Here's how the part is built. I have some questions about the finished solid (model axes, mm). Face numbers are marked on the shaded views. Coordinates: 2 decimals unless noted, no trailing zeros. Write each loop counter-clockwise with the first axis right and the second up, starting at its lowest first coordinate (ties: lowest second). Pieces come first, ordered by that corner, then holes. Notation, with made-up numbers: M -13.75,6.25 L 16.25,6.25 A36 cw 16.25,42.25 Z; hole C 41.5,58 d6. An arc over 180 degrees is marked long. Use one line per item in the form item = value. Start each with the question number.
1. I want a section at C-C, the plane z = 24.75. List the corners of the cut face in (x, y) for me.
2. I want a section at A-A, the plane x = -16. List the corners of the cut face in (y, z) for me.
3. Thinking about a two-plate mould opening in X: for the marked faces 1, 2 and 3, which applies, released by +X, released by -X, zero draft, split by the parting line, or undercut?
4. I want a section at B-B, the plane y = -14.5. List the corners of the cut face in (x, z) for me, plus the area to 3 significant figures.
5. I want a section at D-D, the plane y = 142. List the corners of the cut face in (x, z) for me.
6. I'm going to push flat-ended pins straight in: pin 1 Ø1 at (y, z) = (197, 22) entering from +X; pin 2 Ø12 at (y, z) = (-1.5, 26.5) entering from +X; pin 3 Ø3 at (y, z) = (181.5, 23) entering from +X. Where does each tip first touch, or does it pass through?
7. Please list where these lines run through material, in increasing order: line 1 along Y through (x, z) = (84, 12); line 2 along Y through (x, z) = (67.5, 17.75); line 3 along X through (y, z) = (186, 15). Write a range as [from, to].
from build123d import *

# Parameters (mm, degrees)
SKETCH1_R           = 27.5
BOSS_EXTRUDE1_DEPTH = 30
CHAMFER1_SIZE       = 10


with BuildPart() as part:
    # Sketch1 → Boss-Extrude1 (new body)
    with BuildSketch(Plane.XY):
        with BuildLine():
            Line((92.3, -35.8), (243.373525417, 274.385312067))
            Line((243.373525417, 274.385312067), (224.493722277, 283.580584405))
            ThreePointArc((224.493722277, 283.580584405), (201.609043027, 283.221639878), (180.06339689, 275.500077984))
            ThreePointArc((180.06339689, 275.500077984), (136.851269704, 260.619417011), (91.159540852, 261.61335942))
            ThreePointArc((91.159540852, 261.61335942), (29.078225578, 246.293169038), (1.375741332, 188.661838097))
            ThreePointArc((1.375741332, 188.661838097), (-13.312623389, 114.954388214), (-54.16864079, 51.87252023))
            ThreePointArc((-54.16864079, 51.87252023), (-59.782430884, -45.288640491), (35.270014595, -66.189319912))
            Line((35.270014595, -66.189319912), (92.3, -35.8))
        make_face()
        with Locations((76.373525417, 188.085312067)):
            Circle(SKETCH1_R, mode=Mode.SUBTRACT)
        Circle(SKETCH1_R, mode=Mode.SUBTRACT)
    extrude(amount=BOSS_EXTRUDE1_DEPTH)

    # Chamfer1
    chamfer1_edges = [part.edges().sort_by_distance(p)[0] for p in [
        (167.836762709, 119.292656033, 0),
        (167.836762709, 119.292656033, 30),
    ]]
    chamfer(chamfer1_edges, length=CHAMFER1_SIZE)


solid = part.part
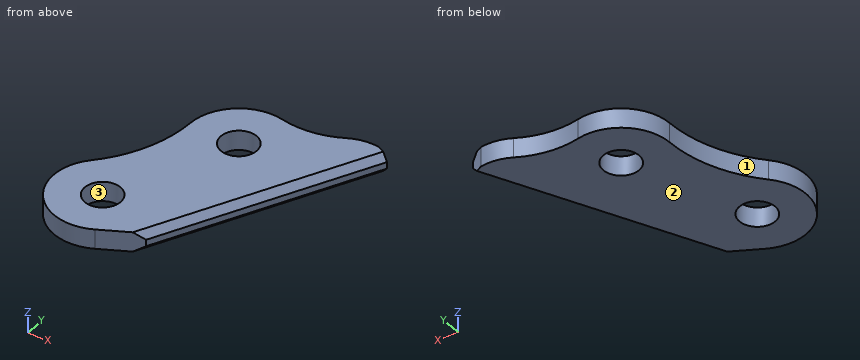
Answer list:
q1.outline = M -54.17,51.87 A75 ccw 35.27,-66.19 L 85.16,-39.6 L 239.1,276.47 L 224.49,283.58 A70 ccw 180.06,275.5 A130 cw 91.16,261.61 A75 ccw 1.38,188.66 A200 cw Z; hole C 0,0 d55; hole C 76.37,188.09 d55
q2.outline = M -73.27,0 L -22.37,0 L -22.37,30 L -73.27,30 Z; M 22.37,0 L 108.65,0 L 108.65,30 L 22.37,30 Z
q3.face_1 = released by -X
q3.face_2 = zero draft
q3.face_3 = undercut
q4.outline = M -73.58,0 L -23.37,0 L -23.37,30 L -73.58,30 Z; M 23.37,0 L 91.55,0 L 102.67,10 L 102.67,20 L 91.55,30 L 23.37,30 Z
q4.area = 3,770 mm²
q5.outline = M -4.51,0 L 167.77,0 L 178.9,10 L 178.9,20 L 167.77,30 L -4.51,30 Z
q6.pin_1 = 204.07
q6.pin_2 = 109.06
q6.pin_3 = 196.62
q7.line_1 = [-40.22, 161.66], [214.51, 262.7]
q7.line_2 = [-49.02, 162.06], [214.11, 262.56]
q7.line_3 = [1.34, 48.95], [103.79, 200.33]
